Verification items for the finished model (mm, model axes). Face numbers are marked on the shaded views. A direction names the side the tool comes from. Coordinates: 2 decimals unless noted, no trailing zeros. Order: outer loops, then holes, each group sorted by start corner. A loop starts at its lowest first (then second) coordinate and runs counter-clockwise, first axis right, second up. Notation, with made-up numbers: M 69,34 L 118,34 A14 ccw 118,41 Z; hole C -10,85 d3. An arc over 180 degrees is marked long. Return JSON: item names as keys, results as strings. Group by question number.
Q1. Section check D-D, the plane z = -20. Enter the section's corners in (x, y), then the cut area to 3 significant figures.
Q2. Thickness scan on probe 1 along Y at (x, z) = (-6, 0); probe 2 along X at (y, z) = (-11.5, -20); probe 3 along Y at (x, z) = (3.5, 0). Record the ranges inside material, lowest first.
Q3. Mould release check, pull along Y, two halves, no side actions. Record for the marked faces 1, 2, 3 and 4: pulls with the +Y half, pulls with the -Y half, needs draft (parallel to the pull), parting line crosses it, or undercut.
Q4. Access from +Z, -Z, +X, -X, +Y, -Y to the whole of each face (thin tool, end or side, straight path). Record for the marked faces 5 and 6.
Q5. Go/stop test with flat-tipped pins: pin 1 Ø2 at (x, y) = (4, -7.5) entering from -Z; pin 2 Ø10 at (x, y) = (-0.5, -7) entering from +Z; pin 3 Ø8 at (x, y) = (-12.5, -10) entering from -Z. Record where each tip stops, or that it passes through.
Q6. Section check A-A, the plane y = 0. Enter the section's corners in (x, z).
Q7. Section check C-C, the plane x = -12.5. Enter the section's corners in (y, z).
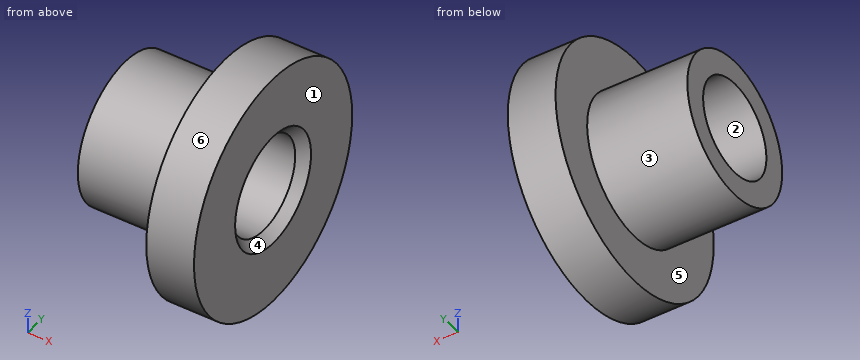
from build123d import *

# Parameters (mm, degrees)
CHAMFER1_SIZE = 2


with BuildPart() as part:
    # Sketch1 → Revolve1 (revolve)
    with BuildSketch(Plane.XY, mode=Mode.PRIVATE) as revolve1_sk:
        Polygon((-20.782396088, 10), (10.217603912, 10), (10.217603912, 25), (0.217603912, 25), (0.217603912, 15), (-20.782396088, 15), align=None)
    revolve(revolve1_sk.sketch.rotate(Axis((-31.662591687, 0, 0), (1, 0, 0)), 90), axis=Axis((-31.662591687, 0, 0), (1, 0, 0)))

    # Chamfer1
    chamfer1_edges = [part.edges().sort_by_distance(p)[0] for p in [
        (10.217603912, 0, -10),
    ]]
    chamfer(chamfer1_edges, length=CHAMFER1_SIZE)


solid = part.part
Numbers:
{
 "1": {"outline": "M 0.22,-15 L 10.22,-15 L 10.22,15 L 0.22,15 Z", "area": "300 mm2"},
 "2": {"probe 1": "y = -15 to -10, 10 to 15", "probe 2": "x = 0.22 to 10.22", "probe 3": "y = -25 to -10, 10 to 25"},
 "3": {"face 1": "needs draft", "face 2": "undercut", "face 3": "parting line crosses it", "face 4": "undercut"},
 "4": {"face 5": "-X", "face 6": "+X, -X"},
 "5": {"pin 1": "stops at z = -24.14", "pin 2": "stops at z = 24.92", "pin 3": "stops at z = -13.75"},
 "6": {"outline": "M -20.78,-15 L 0.22,-15 L 0.22,-25 L 10.22,-25 L 10.22,-12 L 8.22,-10 L -20.78,-10 Z; M -20.78,10 L 8.22,10 L 10.22,12 L 10.22,25 L 0.22,25 L 0.22,15 L -20.78,15 Z"},
 "7": {"outline": "C 0,0 d30; hole C 0,0 d20"}
}
